Input: part model. Units: mm. Frame: model coordinates. A direction names the side the tool comes from. Coordinates: 2 decimals unless noted, no trailing zeros. Write each loop counter-clockwise with the first axis right and the second up, starting at its lowest first coordinate (ties: lowest second). Pieces come first, ordered by that corner, then holes. Notation, with made-up numbers: (-12, 15) - (27, 15) arc R22 ccw to (27, 36) - close; hole circle Ø11 at (-39, 28). An arc over 180 degrees is marked (long way). One line per question, with ' | ' between items. Start each with the question number.
1) Section query A-A on z = 26. Give the number of separate pieces and of enclosed holes in the cut face, and give its area (3 significant figures).
2) First-contact query: P1, Ø12.5, axis at x = 84, y = 120, coming from the -Z side; P2, Ø20, axis at y = 866, z = 21.5, coming from the -X side. Flat tips, straight axial feed; report the tip coordinate or a pass-through.
3) Section query B-B on y = 671.5. Return loops of the section in (x, z).
4) Section query C-C on x = 257. Return loops of the section in (y, z), and give its area (3 significant figures).
5) Line query: line 1 (Y direction, x = 164, z = 30); line 2 (X direction, y = 611.5, z = 14); line 3 (X direction, y = 1090, z = 27.5). Output: solid intervals per line, ascending.
6) Draft query along Y for faces 6 (the flat face through (135, 875, 20)), 7 (the flat face through (85.165, 418.457, 19.72)), 8 (the flat face through (283, 1290, 20)), 9 (the flat face through (197, 654, 40)). Return one class per face: released by +Y, released by -Y, zero draft, split by the parting line, or undercut.
7) Reachability of faces 1 (the flat face through (85.165, 933.457, 19.72)), 2 (the flat face through (154, 59, 20)), 3 (the cylindrical face through (169.645, 658.854, 20.28)), 4 (the flat face through (30, 1061, 20)), 5 (the flat face through (197, 654, 0)) from +Z, -Z, +X, -X, +Y, -Y: full face, straight path, thin tool, end or side. Return the list, or none.
```python
from build123d import *

# Parameters (mm, degrees)
BOSS_EXTRUDE1_DEPTH = 40
CHAMFER1_SIZE       = 160
M24_TAPPED_HOLE1_D  = 21
CUT_EXTRUDE1_DEPTH  = 1351.88896657
FILLET1_R           = 10
SKETCH4_W           = 30
SKETCH4_H           = 822.818816594
CUT_EXTRUDE2_DEPTH  = 1351.88896657
FILLET2_R           = 20
FILLET3_R           = 10


with BuildPart() as part:
    # Sketch1 → Boss-Extrude1 (new body)
    with BuildSketch(Plane.XY):
        Polygon((154, 0), (154, 120), (359, 500), (399, 500), (399, 1290), (0, 1290), (0, 0), align=None)
    extrude(amount=BOSS_EXTRUDE1_DEPTH)

    # Chamfer1
    chamfer1_edges = [part.edges().sort_by_distance(p)[0] for p in [
        (0, 1290, 20),
    ]]
    chamfer(chamfer1_edges, length=CHAMFER1_SIZE)

    # M24 Tapped Hole1 (through all)
    with Locations(Plane(origin=(164, 1090, 0), x_dir=(-1, 0, 0), z_dir=(0, 0, -1))):
        with Locations((0, 0), (0, -440), (80, -970)):
            Hole(M24_TAPPED_HOLE1_D / 2)

    # Sketch3 → Cut-Extrude1 (cut, through all)
    with BuildSketch(Plane(origin=(0, 0, 0), x_dir=(-1, 0, 0), z_dir=(0, 0, -1))):
        Polygon((-135, 835), (0, 785), (0, 965), (-135, 915), align=None)
        Polygon((-135, 400), (-135, 320), (0, 270), (0, 450), align=None)
    extrude(amount=-CUT_EXTRUDE1_DEPTH, mode=Mode.SUBTRACT)

    # Fillet1
    fillet1_edges = [part.edges().sort_by_distance(p)[0] for p in [
        (135, 400, 20),
        (0, 450, 20),
        (0, 270, 20),
        (135, 320, 20),
        (0, 965, 20),
        (0, 785, 20),
        (135, 835, 20),
        (135, 915, 20),
    ]]
    fillet(fillet1_edges, radius=FILLET1_R)

    # Sketch4 → Cut-Extrude2 (cut, through all)
    with BuildSketch(Plane(origin=(0, 0, 0), x_dir=(-1, 0, 0), z_dir=(0, 0, -1))):
        with Locations((-15, 748.590591703)):
            Rectangle(SKETCH4_W, SKETCH4_H)
    extrude(amount=-CUT_EXTRUDE2_DEPTH, mode=Mode.SUBTRACT)

    # Fillet2
    fillet2_edges = [part.edges().sort_by_distance(p)[0] for p in [
        (30, 953.888888889, 20),
        (30, 438.888888889, 20),
        (30, 796.111111111, 20),
    ]]
    fillet(fillet2_edges, radius=FILLET2_R)

    # Fillet3
    fillet3_edges = [part.edges().sort_by_distance(p)[0] for p in [
        (30, 1160, 20),
        (160, 1290, 20),
    ]]
    fillet(fillet3_edges, radius=FILLET3_R)


solid = part.part
```
Answer key:
1) separate pieces: 1 | enclosed holes: 3 | area: 366,000 mm²
2) P1: through | P2: x = 135
3) outline: (30, 0) - (399, 0) - (399, 40) - (30, 40) - close
4) outline: (310.93, 0) - (1290, 0) - (1290, 40) - (310.93, 40) - close | area: 39,200 mm²
5) line 1: 138.54 to 639.5, 660.5 to 1079.5, 1100.5 to 1290 | line 2: 30 to 399 | line 3: 30 to 153.5, 174.5 to 399
6) face 6: undercut | face 7: undercut | face 8: released by +Y | face 9: zero draft
7) face 1: +Z, -Z, -X | face 2: +Z, -Z, +X, -Y | face 3: +Z, -Z | face 4: +Z, -Z, -X, +Y | face 5: -Z, +X, -X, +Y, -Y
